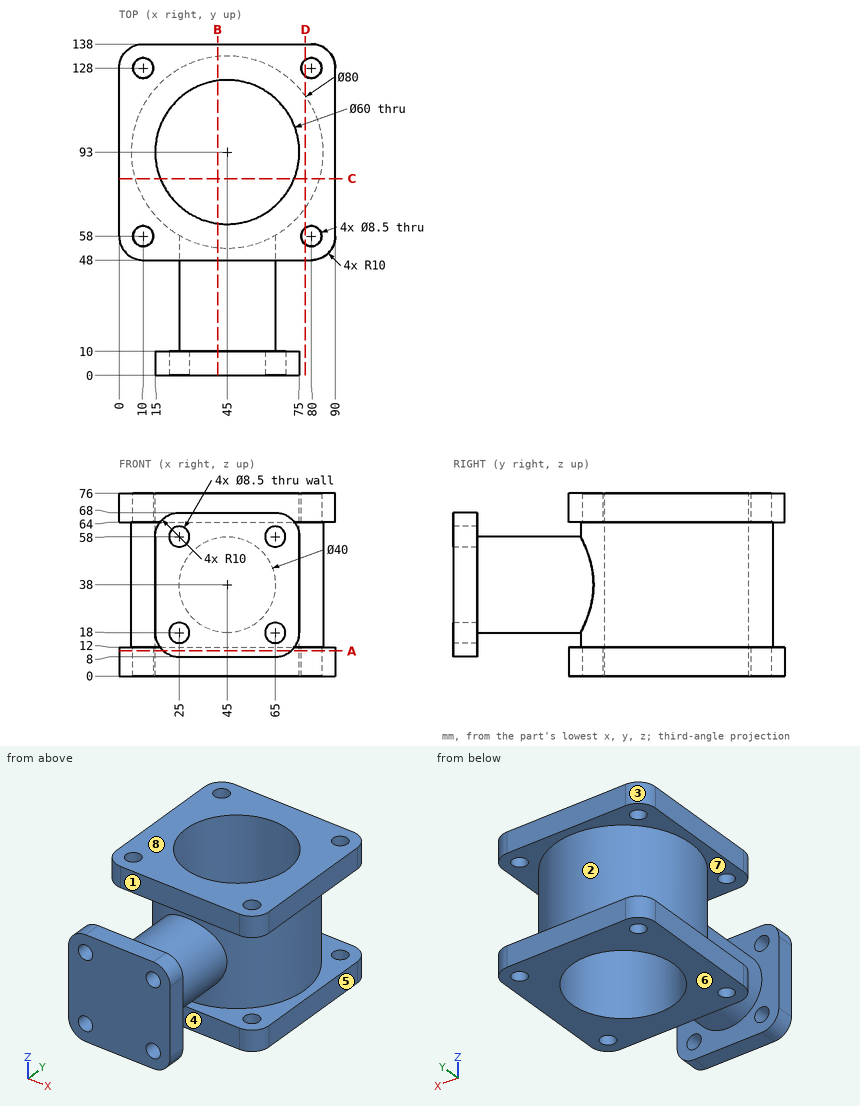
Geometry: see drawing. Coordinates: mm, zero at the bounding-box minimum. A direction names the side the tool comes from. Coordinates: 2 decimals unless noted, no trailing zeros. Order: outer loops, then holes, each group sorted by start corner. A loop starts at its lowest first (then second) coordinate and runs counter-clockwise, first axis right, second up. Notation, with made-up numbers: (-14.75, -23) - (6.25, -23) arc R19 cw to (6.25, -10) - close; hole circle Ø10 at (12, 5.25). An arc over 180 degrees is marked (long way). Use one line per item in the form item = value.
1) Section D-D (x = 77.5). Return loops of the section in (y, z).
Solutions:
outline = (48, 0) - (54.56, 0) - (54.56, 12) - (48, 12) - close; (48, 64) - (54.56, 64) - (54.56, 76) - (48, 76) - close; (61.44, 0) - (124.56, 0) - (124.56, 12) - (116.32, 12) - (116.32, 64) - (124.56, 64) - (124.56, 76) - (61.44, 76) - (61.44, 64) - (69.68, 64) - (69.68, 12) - (61.44, 12) - close; (131.44, 0) - (138, 0) - (138, 12) - (131.44, 12) - close; (131.44, 64) - (138, 64) - (138, 76) - (131.44, 76) - close
2) Ray query, L1, parallel to X at y = 7.75, z = 18; L2, parallel to X at y = 128, z = 7; L3, parallel to Y at x = 10, z = 3.25. Return the intervals inside material, ascending.
Solutions:
L1 = 15 to 20.75, 29.25 to 60.75, 69.25 to 75
L2 = 0 to 5.75, 14.25 to 75.75, 84.25 to 90
L3 = 48 to 53.75, 62.25 to 123.75, 132.25 to 138
3) Section A-A (z = 10.5). Return loops of the section in (x, y).
Solutions:
outline = (0, 58) arc R10 ccw to (10, 48) - (80, 48) arc R10 ccw to (90, 58) - (90, 128) arc R10 ccw to (80, 138) - (10, 138) arc R10 ccw to (0, 128) - close; (18.39, 0) - (71.61, 0) - (71.61, 10) - (18.39, 10) - close; hole circle Ø8.5 at (10, 58); hole circle Ø8.5 at (10, 128); hole circle Ø60 at (45, 93); hole circle Ø8.5 at (80, 58); hole circle Ø8.5 at (80, 128)
4) Mould query, pull axis Z, two halves, no side actions, for the marked faces 5, 6, 7 and 8. Classes: +Z half, -Z half, draft (parallel to the pull), parting line (faces both ways), or undercut.
Solutions:
face_5 = draft
face_6 = -Z half
face_7 = undercut
face_8 = +Z half
5) Section C-C (y = 82). Return loops of the section in (x, z), then the cut area to 3 significant figures.
Solutions:
outline = (0, 0) - (17.09, 0) - (17.09, 76) - (0, 76) - (0, 64) - (6.54, 64) - (6.54, 12) - (0, 12) - close; (72.91, 0) - (90, 0) - (90, 12) - (83.46, 12) - (83.46, 64) - (90, 64) - (90, 76) - (72.91, 76) - close
area = 1,920 mm^2
6) Section B-B (x = 41). Return loops of the section in (y, z), then the cut area to 3 significant figures.
Solutions:
outline = (0, 8) - (10, 8) - (10, 18.4) - (53.2, 18.4) - (53.2, 12) - (48, 12) - (48, 0) - (63.27, 0) - (63.27, 76) - (48, 76) - (48, 64) - (53.2, 64) - (53.2, 57.6) - (10, 57.6) - (10, 68) - (0, 68) - close; (122.73, 0) - (138, 0) - (138, 12) - (132.8, 12) - (132.8, 64) - (138, 64) - (138, 76) - (122.73, 76) - close
area = 4,070 mm^2
7) Pin query (flat end, axial travel): pin 1 (11 mm diameter, centred on x = 65, z = 18, fed in from +Y); pin 2 (7 mm diameter, centred on x = 25, z = 18, fed in from -Y); pin 3 (10 mm diameter, centred on x = 64, z = 63.5, fed in from +Y); pin 4 (11 mm diameter, centred on y = 3, z = 33, fed in from -X). Return the tip coordinate at first contact, or that it passes through.
Solutions:
pin_1 = 130.28
pin_2 = 56.56
pin_3 = 138
pin_4 = 15
8) Set-up query: the marked faces 1, 2, 3 and 4. Return all of +Z, -Z, +X, -X, +Y, -Y with unobstructed straight access to the full face (end or side cutting, diameter ignored); none if empty.
Solutions:
face_1 = +Z, +X, -X
face_2 = none
face_3 = +Z, -Z, -X, +Y
face_4 = -Z, +X, -X
